Build history of the part. All positions in model axes, mm. A direction names the side the tool comes from. Give positions to 0.01 mm unless a question says otherwise; leave off trailing zeros. Order: outer loops, then holes, each group sorted by start corner. A loop starts at its lowest first (then second) coordinate and runs counter-clockwise, first axis right, second up. Notation, with made-up numbers: (30.5, 54) - (81.5, 54) arc R24 cw to (81.5, 66) - close; hole circle Ø6 at (34, 89). An arc over 180 degrees is marked (long way). Write each question's results on one line, items separated by ' | '. Start each with the question number.
1) Cut at A-A on z = 3.75. List the corners of the cut face in (x, y).
2) Cut at B-B on x = 65. List the corners of the cut face in (y, z).
3) Drill centre lines: line 1 along Z through (x, y) = (48.5, 10); line 2 along Y through (x, z) = (72.5, -4.75); line 3 along Y through (x, z) = (65, 9.15). Where is each one in solid material? Low to high. Write a range as from..to.
4) Drop flat-ended pins along their axis: pin 1 Ø9.5 at (x, y) = (70, 6.5) entering from -Z; pin 2 Ø17 at (x, y) = (65, 0) entering from -Z. Give the stop position or say it passes through.
5) Cut at C-C on z = -6.25. List the corners of the cut face in (x, y).
6) Cut at D-D on y = 13. List the corners of the cut face in (x, z).
7) Two-plate mould, pull along X, no slides. Class faces 1 (the face through (59, 22.5, 0)), 2 (the face through (56.376, -5.07, -8.035)), 3 (the face through (95, 0, 7)): +X half, -X half, draft (parallel to the pull), parting line (faces both ways), or undercut.
8) Tool access for faces 4 (the face through (73.624, 5.07, -8.035)), 5 (the face through (60, -22.5, 0)), 6 (the face through (61, -15.5, 0)): list every direction of +Z, -Z, +X, -X, +Y, -Y with a clear straight run to the whole face (end or side of a thin tool).
from build123d import *

# Parameters (mm, degrees)
EXTRUDE_1_DEPTH     = 10.5
SKETCH_2_W          = 11
SKETCH_2_H          = 31
CUT_EXTRUDE_1_DEPTH = 75.76938691
CUT_EXTRUDE_2_REACH = 101.861
SKETCH_3_R          = 6.5
CUT_EXTRUDE_5_REACH = 101.861
SKETCH_4_R          = 6.5


with BuildPart() as part:
    # 草图1 → 凸台-拉伸1 (new, symmetric)
    with BuildSketch(Plane.XY):
        with BuildLine():
            Line((95, 22.5), (95, -22.5))
            Line((95, -22.5), (24.473684211, -22.5))
            Line((24.473684211, -22.5), (24.473684211, -17.350469191))
            ThreePointArc((24.473684211, -17.350469191), (30, 0), (24.473684211, 17.350469191))
            Line((24.473684211, 17.350469191), (24.473684211, 22.5))
            Line((24.473684211, 22.5), (95, 22.5))
        make_face()
    extrude(amount=EXTRUDE_1_DEPTH, both=True)

    # 草图2 → 切除-拉伸1 (cut, through all)
    with BuildSketch(Plane(origin=(95, 0, 0), x_dir=(0, 0, -1), z_dir=(1, 0, 0))):
        Rectangle(SKETCH_2_W, SKETCH_2_H)
    extrude(amount=-CUT_EXTRUDE_1_DEPTH, mode=Mode.SUBTRACT)

    # 草图3 → 切除-拉伸2 (cut, up to next)
    with BuildSketch(Plane.XY.offset(10.5), mode=Mode.PRIVATE) as cut_extrude_2_sk1:
        with Locations((65, 0)):
            Circle(SKETCH_3_R)
    cut_extrude_2_tool1 = extrude(cut_extrude_2_sk1.sketch, amount=-CUT_EXTRUDE_2_REACH, mode=Mode.PRIVATE) & part.part
    add(cut_extrude_2_tool1.solids().sort_by_distance((65, 0, 10.5))[0], mode=Mode.SUBTRACT)

    # 草图4 → 切除-拉伸5 (cut, up to next)
    with BuildSketch(Plane(origin=(0, 0, -10.5), x_dir=(-1, 0, 0), z_dir=(0, 0, -1)), mode=Mode.PRIVATE) as cut_extrude_5_sk1:
        Polygon((-76.55, 0), (-70.779489597, -10), (-59.220510403, -10), (-53.45, 0), (-59.220510403, 10), (-70.779489597, 10), align=None)
        with Locations(Location((-65, 0, 0), (0, 0, 180))):
            Circle(SKETCH_4_R, mode=Mode.SUBTRACT)
    cut_extrude_5_tool1 = extrude(cut_extrude_5_sk1.sketch, amount=-CUT_EXTRUDE_5_REACH, mode=Mode.PRIVATE) & part.part
    # 草图4 → 切除-拉伸5 (cut, up to next)
    with BuildSketch(Plane(origin=(0, 0, -10.5), x_dir=(-1, 0, 0), z_dir=(0, 0, -1)), mode=Mode.PRIVATE) as cut_extrude_5_sk2:
        with Locations(Location((-65, 0, 0), (0, 0, 180))):
            Circle(SKETCH_4_R)
    cut_extrude_5_tool2 = extrude(cut_extrude_5_sk2.sketch, amount=-CUT_EXTRUDE_5_REACH, mode=Mode.PRIVATE) & part.part
    add(cut_extrude_5_tool1.solids().sort_by_distance((73.400096, -4.847284, -10.5))[0], mode=Mode.SUBTRACT)
    add(cut_extrude_5_tool2.solids().sort_by_distance((65, 0, -10.5))[0], mode=Mode.SUBTRACT)


solid = part.part
Results:
1) outline: (24.47, -22.5) - (95, -22.5) - (95, -15.5) - (25.69, -15.5) arc R30 cw to (24.47, -17.35) - close; (24.47, 17.35) arc R30 cw to (25.69, 15.5) - (95, 15.5) - (95, 22.5) - (24.47, 22.5) - close
2) outline: (-22.5, -10.5) - (-10, -10.5) - (-10, -5.5) - (-15.5, -5.5) - (-15.5, 5.5) - (-6.5, 5.5) - (-6.5, 10.5) - (-22.5, 10.5) - close; (6.5, 5.5) - (15.5, 5.5) - (15.5, -5.5) - (10, -5.5) - (10, -10.5) - (22.5, -10.5) - (22.5, 10.5) - (6.5, 10.5) - close
3) line 1: -10.5..-5.5, 5.5..10.5 | line 2: -22.5..-15.5, 15.5..22.5 | line 3: -22.5..-6.5, 6.5..22.5
4) pin 1: z = -10.5 | pin 2: z = 5.5
5) outline: (24.47, -22.5) - (95, -22.5) - (95, 22.5) - (24.47, 22.5) - (24.47, 17.35) arc R30 cw to (24.47, -17.35) - close; hole (53.45, 0) - (59.22, -10) - (70.78, -10) - (76.55, 0) - (70.78, 10) - (59.22, 10) - close
6) outline: (27.04, -10.5) - (95, -10.5) - (95, -5.5) - (27.04, -5.5) - close; (27.04, 5.5) - (95, 5.5) - (95, 10.5) - (27.04, 10.5) - close
7) face 1: draft | face 2: undercut | face 3: +X half
8) face 4: -Z | face 5: +Z, -Z, +X, -X, -Y | face 6: +X, -X
